CAD build for the part. Positions are in the model's coordinates, mm. A direction names the side the tool comes from. Give positions to 0.01 mm unless a question says otherwise; leave off trailing zeros. Write each loop counter-clockwise with the first axis right and the second up, starting at its lowest first coordinate (ties: lowest second). Pieces come first, ordered by that corner, then holes. Notation, with made-up numbers: M 86,0.5 L 104,0.5 A18 ccw 104,9.5 Z; hole C 85.5,67 d10. An arc over 180 degrees is marked long. One line per question, with ' | ' between items. Start each with the question number.
1. Cut at A-A, the plane x = -13. Count the separate pieces of the cut face and the enclosed holes in it, then the cut area to 3 significant figures.
2. Flat gauge pins, fed straight in: pin 1 (5 mm diameter, centred on y = -30.5, z = -61, fed in from +X); pin 2 (4 mm diameter, centred on y = 874.5, z = -97.5, fed in from -X); pin 3 (2 mm diameter, centred on y = -1093.5, z = 164, fed in from -X). Where does each tip first touch, or does it go through?
3. Cut at C-C, the plane y = 608. Write the cut outline in (x, z).
4. Which spindle directions (+Z, -Z, +X, -X, +Y, -Y) get a long thin tool onto all of the face, cutting with end or side? Do faces 1 (the face through (-2, -993, 6)), 2 (the face through (-38, -811, 6)), 3 (the face through (-18, 868, 6)). Say none if no direction does.
5. Wall check: L1, parallel to Y at x = -35, z = -335; L2, parallel to X at y = -315, z = -21.5; L3, parallel to X at y = -26.5, z = -313. Give the ranges that are in metal, low to high.
6. Pull direction Y, two halves, no side cores. Call faces 4 (the face through (0, -410, 6)), 5 (the face through (-20.25, 753.77, 5.79)), 6 (the face through (-19.75, 868.98, 5.79)): released by +Y, released by -Y, zero draft, split by the parting line, or undercut.
```python
from build123d import *

# Parameters (mm, degrees)
EXTRUDE_THIN1_DEPTH = 413.5


with BuildPart() as part:
    # Sketch1 → Extrude-Thin1 (new, symmetric)
    with BuildSketch(Plane.XY):
        Polygon((-30, -1095), (0, -1095), (0, -895), (-36, -841), (-36, -781), (0, -727), (0, -84), (-36, -30), (-36, 30), (0, 84), (0, 727), (-36, 781), (-36, 841), (0, 895), (0, 1095), (-30, 1095), (-30, 1093), (-2, 1093), (-2, 895.605551275), (-38, 841.605551275), (-38, 780.394448725), (-2, 726.394448725), (-2, 84.605551275), (-38, 30.605551275), (-38, -30.605551275), (-2, -84.605551275), (-2, -726.394448725), (-38, -780.394448725), (-38, -841.605551275), (-2, -895.605551275), (-2, -1093), (-30, -1093), align=None)
    extrude(amount=EXTRUDE_THIN1_DEPTH, both=True)


solid = part.part
```
Here are the results:
1) separate pieces: 8 | enclosed holes: 0 | area: 21,200 mm^2
2) pin 1: x = -34 | pin 2: x = -17.4 | pin 3: x = -30
3) outline: M -2,-413.5 L 0,-413.5 L 0,413.5 L -2,413.5 Z
4) face 1: +Z, -Z, -X | face 2: +Z, -Z, -X, +Y, -Y | face 3: +Z, -Z, +X
5) L1: -846.11 to -842.5, -779.5 to -775.89, -35.11 to -31.5, 31.5 to 35.11, 775.89 to 779.5, 842.5 to 846.11 | L2: -2 to 0 | L3: -38 to -36
6) face 4: zero draft | face 5: undercut | face 6: undercut
